from build123d import *


with BuildPart() as part:
    # Sketch1 → Revolve1 (revolve)
    with BuildSketch(Plane.XY.offset(-440.692981355), mode=Mode.PRIVATE) as revolve1_sk:
        Polygon((551.230642584, 721.895595987), (551.230642584, 804.895595987), (556.230642584, 804.895595987), (556.230642584, 819.895595987), (581.230642584, 819.895595987), (581.230642584, 831.895595987), (558.230642584, 831.895595987), (558.230642584, 846.895595987), (547.230642584, 846.895595987), (547.230642584, 816.895595987), (541.230642584, 816.895595987), (541.230642584, 701.895595987), (547.230642584, 701.895595987), (547.230642584, 681.895595987), (556.230642584, 681.895595987), (556.230642584, 721.895595987), align=None)
    revolve(revolve1_sk.sketch.rotate(Axis((521.230642584, 846.895595987, -440.692981355), (0, -1, 0)), 270), axis=Axis((521.230642584, 846.895595987, -440.692981355), (0, -1, 0)))


solid = part.part
Here's how the part is built. I have some questions about the finished solid (model axes, mm). A direction names the side the tool comes from. Give positions to 0.01 mm unless a question says otherwise; leave off trailing zeros. Loops run counter-clockwise (first coordinate to the right, second up) from the corner with the lowest first, then second, coordinate; pieces in that order, holes last. Notation, with made-up numbers: (82.5, 72.25) -> (131.5, 72.25) arc R30 ccw to (131.5, 110.25) -> close; hole circle Ø1 at (-15, -39). An arc over 180 degrees is marked (long way). Answer as a JSON object with one key per item and string values. Group by question number.
Item 1: Imagine slicing it at C-C on y = 813. Write out the boundary of the cut face in (x, z).
Item 2: I need wall thicknesses on L1, parallel to Y at x = 493, z = -476; L2, parallel to X at y = 728.5, z = -455.5; L3, parallel to Y at x = 490.5, z = -441. Which ranges of each line are inside material? Lowest first, please.
Item 3: Will these pins go through, and if not, where does the flat tip stop? pin 1 (12 mm diameter, centred on x = 493.5, y = 703.5, fed in from +Z); pin 2 (8 mm diameter, centred on x = 517, y = 828, fed in from -Z); pin 3 (12 mm diameter, centred on y = 743, z = -408.5, fed in from +X).
Item 4: On a 3-axis mill with a long thin cutter (end or side, diameter ignored), from which of +Z, -Z, +X, -X, +Y, -Y can I reach the whole of each face in a straight line? I mean faces 5 (the cylindrical face through (547.01, 831.69, -437.31)), 6 (the cylindrical face through (547.01, 691.76, -437.31)), 7 (the flat face through (536.9, 804.896, -414.9)). Say none if no direction works.
Item 5: Imagine slicing it at D-D on z = -401. Write out the boundary of the cut face in (x, y), then the cut area to 3 significant figures.
Item 6: Thinking about a two-plate mould opening in Y: for faces 1 (the cylindrical face through (490.18, 812.5, -456.84)), 2 (the flat face through (506, 701.896, -427)), 3 (the flat face through (495, 831.896, -413)), 4 (the cylindrical face through (550.975, 763.977, -436.788)), which applies, pulls with the +Y half, pulls with the -Y half, needs draft (parallel to the pull), parting line crosses it, or undercut?
Answer list:
{
 "1": {"outline": "circle Ø70 at (521.23, -440.69); hole circle Ø40 at (521.23, -440.69)"},
 "2": {"L1": "y = 819.9 to 831.9", "L2": "x = 495.14 to 507.79, 534.68 to 547.32", "L3": "y = 681.9 to 721.9, 804.9 to 846.9"},
 "3": {"pin 1": "stops at z = -413.26", "pin 2": "stops at z = -500.69", "pin 3": "stops at x = 535.86"},
 "4": {"face 5": "+Y", "face 6": "-Y", "face 7": "none"},
 "5": {"outline": "(476.24, 819.9) -> (566.22, 819.9) -> (566.22, 831.9) -> (476.24, 831.9) -> close", "area": "1,080 mm2"},
 "6": {"face 1": "needs draft", "face 2": "pulls with the -Y half", "face 3": "pulls with the +Y half", "face 4": "undercut"}
}
